Verification items for the finished model (mm, model axes). A direction names the side the tool comes from. Give positions to 0.01 mm unless a question says otherwise; leave off trailing zeros. Write each loop counter-clockwise with the first axis right and the second up, starting at its lowest first coordinate (ties: lowest second). Pieces come first, ordered by that corner, then holes. Notation, with made-up numbers: (85.25, 39) -> (108.25, 39) arc R21 cw to (108.25, 76) -> close; hole circle Ø8 at (53, 50). An arc over 180 degrees is marked (long way). Answer as CSV lines item,"result". Start each with the question number.
1) Tool access check on faces 1 (the flat face through (135, 12, 3)), 2 (the flat face through (180, -66, 2)), 3 (the flat face through (22, 0, 2)). Record the directions out of +Z, -Z, +X, -X, +Y, -Y that give a thin tool (end or side, any length) a straight path to the whole face; none if there is none.
2) Sectioned sample at A-A on z = 1.9. Record the cut outline in (x, y).
3) Material ranges on L1, parallel to Y at x = 40, z = 4.75; L2, parallel to X at y = 2, z = 3.15, recorded low to high.
4) Sectioned sample at C-C on x = 163. Record the cut outline in (y, z), and give its area (3 significant figures).
5) Sectioned sample at B-B on y = 10.5. Record the cut outline in (x, z), and give its area (3 significant figures).
```python
from build123d import *

# Parameters (mm, degrees)
SKETCH_1_W      = 180
SKETCH_1_H      = 130
EXTRUDE_1_DEPTH = 5
SKETCH_2_W      = 90
SKETCH_2_H      = 5
EXTRUDE_2_DEPTH = 25


with BuildPart() as part:
    # 草图1 → 凸台-拉伸1 (new body)
    with BuildSketch(Plane.XY):
        with Locations((90, -65)):
            Rectangle(SKETCH_1_W, SKETCH_1_H)
    extrude(amount=EXTRUDE_1_DEPTH)

    # 草图2 → 凸台-拉伸2 (add)
    with BuildSketch(Plane(origin=(0, 0, 0), x_dir=(1, 0, 0), z_dir=(0, 1, 0))):
        with Locations((90, -2.5)):
            Rectangle(SKETCH_2_W, SKETCH_2_H)
    extrude(amount=EXTRUDE_2_DEPTH)


solid = part.part
```
Ans:
1,face 1,"+Z, -Z, +X, +Y"
1,face 2,"+Z, -Z, +X, +Y, -Y"
1,face 3,"+Z, -Z, -X, +Y"
2,outline,"(0, -130) -> (180, -130) -> (180, 0) -> (135, 0) -> (135, 25) -> (45, 25) -> (45, 0) -> (0, 0) -> close"
3,L1,"y = -130 to 0"
3,L2,"x = 45 to 135"
4,outline,"(-130, 0) -> (0, 0) -> (0, 5) -> (-130, 5) -> close"
4,area,"650 mm²"
5,outline,"(45, 0) -> (135, 0) -> (135, 5) -> (45, 5) -> close"
5,area,"450 mm²"
